Here's how the part is built. I have some questions about the finished solid (model axes, mm). Face numbers are marked on the shaded views. A direction names the side the tool comes from. Coordinates: 2 decimals unless noted, no trailing zeros. Loops run counter-clockwise (first coordinate to the right, second up) from the corner with the lowest first, then second, coordinate; pieces in that order, holes last. Notation, with made-up numbers: (60.5, -35) - (79.5, -35) arc R14 ccw to (79.5, -31) - close; hole circle Ø7 at (61.25, 13). An arc over 180 degrees is marked (long way). Use a Markdown table: item, result.
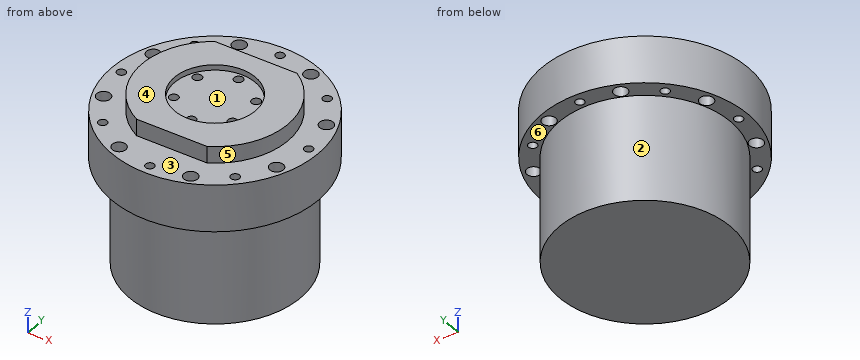
```python
from build123d import *

# Parameters (mm, degrees)
SKETCH1_R           = 1.66
BOSS_EXTRUDE1_DEPTH = 6.2
SKETCH2_R           = 38.25
SKETCH2_R_2         = 1.6
SKETCH2_R_3         = 2.5
BOSS_EXTRUDE2_DEPTH = 17.5
SKETCH3_R           = 31.75
BOSS_EXTRUDE3_DEPTH = 39.3
SKETCH4_R           = 15
CUT_EXTRUDE1_DEPTH  = 2


with BuildPart() as part:
    # Sketch1 → Boss-Extrude1 (new body)
    with BuildSketch(Plane.XY):
        with BuildLine():
            Line((-15.516105129, 22.096390692), (14.325275898, 22.886381768))
            ThreePointArc((14.325275898, 22.886381768), (26.994312242, -0.554171996), (13.373923279, -23.455024539))
            Line((13.373923279, -23.455024539), (-12.114210645, -24.129772076))
            ThreePointArc((-12.114210645, -24.129772076), (-26.927181778, -1.981636062), (-15.516105129, 22.096390692))
        make_face()
        with Locations(Location((0, 12.5, 0), (0, 0, 180))):
            Circle(SKETCH1_R, mode=Mode.SUBTRACT)
        with Locations(Location((10.825317547, 6.25, 0), (0, 0, 180))):
            Circle(SKETCH1_R, mode=Mode.SUBTRACT)
        with Locations(Location((0, -12.5, 0), (0, 0, 180))):
            Circle(SKETCH1_R, mode=Mode.SUBTRACT)
        with Locations(Location((10.825317547, -6.25, 0), (0, 0, 180))):
            Circle(SKETCH1_R, mode=Mode.SUBTRACT)
        with Locations(Location((-10.825317547, -6.25, 0), (0, 0, 180))):
            Circle(SKETCH1_R, mode=Mode.SUBTRACT)
        with Locations(Location((-10.825317547, 6.25, 0), (0, 0, 180))):
            Circle(SKETCH1_R, mode=Mode.SUBTRACT)
    extrude(amount=BOSS_EXTRUDE1_DEPTH)

    # Sketch2 → Boss-Extrude2 (add)
    with BuildSketch(Plane(origin=(0, 0, 0), x_dir=(-1, 0, 0), z_dir=(0, 0, -1))):
        Circle(SKETCH2_R)
        with Locations((0, 34.5)):
            Circle(SKETCH2_R_2, mode=Mode.SUBTRACT)
        with Locations(Location((24.395183951, 24.395183951, 0), (0, 0, 180))):
            Circle(SKETCH2_R_2, mode=Mode.SUBTRACT)
        with Locations((34.5, 0)):
            Circle(SKETCH2_R_2, mode=Mode.SUBTRACT)
        with Locations(Location((24.395183951, -24.395183951, 0), (0, 0, 180))):
            Circle(SKETCH2_R_2, mode=Mode.SUBTRACT)
        with Locations(Location((0, -34.5, 0), (0, 0, 180))):
            Circle(SKETCH2_R_2, mode=Mode.SUBTRACT)
        with Locations((-24.395183951, -24.395183951)):
            Circle(SKETCH2_R_2, mode=Mode.SUBTRACT)
        with Locations(Location((-34.5, 0, 0), (0, 0, 180))):
            Circle(SKETCH2_R_2, mode=Mode.SUBTRACT)
        with Locations((-24.395183951, 24.395183951)):
            Circle(SKETCH2_R_2, mode=Mode.SUBTRACT)
        with Locations((13.202578417, 31.873843872)):
            Circle(SKETCH2_R_3, mode=Mode.SUBTRACT)
        with Locations(Location((31.873843872, 13.202578417, 0), (0, 0, 180))):
            Circle(SKETCH2_R_3, mode=Mode.SUBTRACT)
        with Locations((31.873843872, -13.202578417)):
            Circle(SKETCH2_R_3, mode=Mode.SUBTRACT)
        with Locations(Location((13.202578417, -31.873843872, 0), (0, 0, 180))):
            Circle(SKETCH2_R_3, mode=Mode.SUBTRACT)
        with Locations((-31.873843872, -13.202578417)):
            Circle(SKETCH2_R_3, mode=Mode.SUBTRACT)
        with Locations(Location((-31.873843872, 13.202578417, 0), (0, 0, 180))):
            Circle(SKETCH2_R_3, mode=Mode.SUBTRACT)
        with Locations((-13.202578417, 31.873843872)):
            Circle(SKETCH2_R_3, mode=Mode.SUBTRACT)
        with Locations(Location((-13.202578417, -31.873843872, 0), (0, 0, 180))):
            Circle(SKETCH2_R_3, mode=Mode.SUBTRACT)
    extrude(amount=BOSS_EXTRUDE2_DEPTH)

    # Sketch3 → Boss-Extrude3 (add)
    with BuildSketch(Plane(origin=(0, 0, -17.5), x_dir=(-1, 0, 0), z_dir=(0, 0, -1))):
        Circle(SKETCH3_R)
    extrude(amount=BOSS_EXTRUDE3_DEPTH)

    # Sketch4 → Cut-Extrude1 (cut)
    with BuildSketch(Plane.XY.offset(6.2)):
        Circle(SKETCH4_R)
    extrude(amount=-CUT_EXTRUDE1_DEPTH, mode=Mode.SUBTRACT)


solid = part.part
```
Q1. Please list where these lines run through material, in increasing order: L1, parallel to Y at x = 0, z = 1.75; L2, parallel to Y at x = 12, z = -16.5; L3, parallel to X at y = 24, z = -10. Write a range as from..to.
Check values:
| item | result |
|---|---|
| L1 | -23.81..-14.16, -10.84..10.84, 14.16..22.51 |
| L2 | -36.32..-34.07, -29.68..29.68, 34.07..36.32 |
| L3 | -29.78..-25.95, -22.84..22.84, 25.95..29.78 |
Q2. Will these pins go through, and if not, where does the flat tip stop? P1, Ø1.7, axis at x = -0.5, y = -13, coming from the +Z side; P2, Ø3, axis at x = -34.5, y = 0, coming from the -Z side; P3, Ø12, axis at y = 15, z = -30, coming from the -X side; P4, Ø10, axis at y = 7.5, z = -5, coming from the +X side.
Check values:
| item | result |
|---|---|
| P1 | z = 0 |
| P2 | through |
| P3 | x = -30.45 |
| P4 | x = 38.17 |
Q3. Which directions (+Z, -Z, +X, -X, +Y, -Y) give clear straight access to the entire face, cutting with the end or side of a thin tool? Please do the marked faces 4, 5 and 6.
Check values:
| item | result |
|---|---|
| face 4 | +Z, +X, -X, +Y, -Y |
| face 5 | +Z, +X |
| face 6 | -Z |
Q4. I want a section at C-C, the plane y = 17.5. Write out the boundary of the cut face in (x, z).
Check values:
| item | result |
|---|---|
| outline | (-34.01, -17.5) - (-26.49, -17.5) - (-26.49, -56.8) - (26.49, -56.8) - (26.49, -17.5) - (34.01, -17.5) - (34.01, 0) - (20.56, 0) - (20.56, 6.2) - (-20.56, 6.2) - (-20.56, 0) - (-34.01, 0) - close |
Q5. I want a section at B-B, the plane z = -16. Give the number of separate pieces and of enclosed holes in the cut face, then the cut area to 3 significant figures.
Check values:
| item | result |
|---|---|
| separate pieces | 1 |
| enclosed holes | 16 |
| area | 4,370 mm^2 |
Q6. If we mould it in two halves opening along X, with no side actions, what happens to the marked faces 1, 2 and 3? For each: pulls with the +X half, pulls with the -X half, needs draft (parallel to the pull), parting line crosses it, or undercut.
Check values:
| item | result |
|---|---|
| face 1 | undercut |
| face 2 | parting line crosses it |
| face 3 | needs draft |
Q7. I want a section at D-D, the plane x = -4.5. Write out the boundary of the cut face in (y, z), then the cut area to 3 significant figures.
Check values:
| item | result |
|---|---|
| outline | (-37.98, -17.5) - (-31.43, -17.5) - (-31.43, -56.8) - (31.43, -56.8) - (31.43, -17.5) - (37.98, -17.5) - (37.98, 0) - (22.39, 0) - (22.39, 6.2) - (14.31, 6.2) - (14.31, 4.2) - (-14.31, 4.2) - (-14.31, 6.2) - (-23.93, 6.2) - (-23.93, 0) - (-37.98, 0) - close |
| area | 4,030 mm^2 |
Q8. I want a section at A-A, the plane y = 0. Write out the boundary of the cut face in (x, z).
Check values:
| item | result |
|---|---|
| outline | (-38.25, -17.5) - (-36.1, -17.5) - (-36.1, 0) - (-38.25, 0) - close; (-32.9, -17.5) - (-31.75, -17.5) - (-31.75, -56.8) - (31.75, -56.8) - (31.75, -17.5) - (32.9, -17.5) - (32.9, 0) - (27, 0) - (27, 6.2) - (15, 6.2) - (15, 4.2) - (-15, 4.2) - (-15, 6.2) - (-27, 6.2) - (-27, 0) - (-32.9, 0) - close; (36.1, -17.5) - (38.25, -17.5) - (38.25, 0) - (36.1, 0) - close |
